Part model, mm, in its own coordinate system. Round coordinates to 2 decimals unless told otherwise and drop trailing zeros. Loops run counter-clockwise (first coordinate to the right, second up) from the corner with the lowest first, then second, coordinate; pieces in that order, holes last. Notation, with made-up numbers: (-6.5, -15) -> (48.5, -15) arc R13 ccw to (48.5, -6) -> close; hole circle Ø2 at (-17.75, -16.5). An arc over 180 degrees is marked (long way). Answer as a JSON object with one key per item and string values. Group by question number.
from build123d import *

# Parameters (mm, degrees)
SKETCH1_W           = 200
SKETCH1_H           = 140
BOSS_EXTRUDE1_DEPTH = 14
CHAMFER1_SIZE       = 5
SKETCH3_R           = 6.5
CUT_EXTRUDE2_DEPTH  = 245.532206468
FILLET1_R           = 10


with BuildPart() as part:
    # Sketch1 → Boss-Extrude1 (new body)
    with BuildSketch(Plane.XY):
        with Locations((100, 70)):
            Rectangle(SKETCH1_W, SKETCH1_H)
    extrude(amount=BOSS_EXTRUDE1_DEPTH)

    # Chamfer1
    chamfer1_edges = [part.edges().sort_by_distance(p)[0] for p in [
        (100, 140, 14),
        (100, 140, 0),
    ]]
    chamfer(chamfer1_edges, length=CHAMFER1_SIZE)

    # Sketch3 → Cut-Extrude2 (cut, through all)
    with BuildSketch(Plane(origin=(0, 0, 0), x_dir=(-1, 0, 0), z_dir=(0, 0, -1))):
        with Locations((-185, 16)):
            Circle(SKETCH3_R)
        with Locations((-100, 16)):
            Circle(SKETCH3_R)
        with Locations((-15, 16)):
            Circle(SKETCH3_R)
    extrude(amount=-CUT_EXTRUDE2_DEPTH, mode=Mode.SUBTRACT)

    # Fillet1
    fillet1_edges = [part.edges().sort_by_distance(p)[0] for p in [
        (200, 0, 7),
        (0, 0, 7),
    ]]
    fillet(fillet1_edges, radius=FILLET1_R)


solid = part.part
Item 1: Drill centre lines: line 1 (X direction, y = 10.5, z = 2.5); line 2 (Y direction, x = 185, z = 6); line 3 (X direction, y = 12, z = 12). Where is each one in solid material? Low to high.
Item 2: Band-saw the part on A-A, the plane y = 16. List the corners of the cut face in (x, z), plus the area to 3 significant figures.
Item 3: Band-saw the part on B-B, the plane x = 100. List the corners of the cut face in (y, z).
Item 4: Two-plate mould, pull along Y, no slides. Class faces 1 (the face through (99, 68, 0)), 2 (the face through (21.494, 16.286, 6.902)), 3 (the face through (99, 137, 2)), 4 (the face through (196.99, 2.85, 7.1)): pulls with the +Y half, pulls with the -Y half, needs draft (parallel to the pull), parting line crosses it, or undercut.
Item 5: Band-saw the part on C-C, the plane z = 2.75. List the corners of the cut face in (x, y).
Entries:
{
 "1": {"line 1": "0 to 11.54, 18.46 to 96.54, 103.46 to 181.54, 188.46 to 200", "line 2": "0 to 9.5, 22.5 to 140", "line 3": "0 to 9.88, 20.12 to 94.88, 105.12 to 179.88, 190.12 to 200"},
 "2": {"outline": "(0, 0) -> (8.5, 0) -> (8.5, 14) -> (0, 14) -> close; (21.5, 0) -> (93.5, 0) -> (93.5, 14) -> (21.5, 14) -> close; (106.5, 0) -> (178.5, 0) -> (178.5, 14) -> (106.5, 14) -> close; (191.5, 0) -> (200, 0) -> (200, 14) -> (191.5, 14) -> close", "area": "2,250 mm²"},
 "3": {"outline": "(0, 0) -> (9.5, 0) -> (9.5, 14) -> (0, 14) -> close; (22.5, 0) -> (135, 0) -> (140, 5) -> (140, 9) -> (135, 14) -> (22.5, 14) -> close"},
 "4": {"face 1": "needs draft", "face 2": "undercut", "face 3": "pulls with the +Y half", "face 4": "pulls with the -Y half"},
 "5": {"outline": "(0, 10) arc R10 ccw to (10, 0) -> (190, 0) arc R10 ccw to (200, 10) -> (200, 137.75) -> (0, 137.75) -> close; hole circle Ø13 at (15, 16); hole circle Ø13 at (100, 16); hole circle Ø13 at (185, 16)"}
}
